Model file for the job. Use its own axes, mm. A direction names the side the tool comes from. Coordinates: 2 decimals unless noted, no trailing zeros. Loops run counter-clockwise (first coordinate to the right, second up) from the corner with the lowest first, then second, coordinate; pieces in that order, holes last. Notation, with made-up numbers: (21.5, 29.5) - (68.5, 29.5) arc R31 ccw to (68.5, 65.5) - close; hole circle Ø8 at (16.25, -38.75). An arc over 180 degrees is marked (long way). Write each question's results on one line, items separated by ' | '. Start each with the question number.
```python
from build123d import *

# Parameters (mm, degrees)
BOSS_EXTRUDE1_DEPTH = 32
SKETCH2_R           = 2.1
CUT_EXTRUDE1_DEPTH  = 35.76550014
SKETCH3_R           = 1.740904785
BOSS_EXTRUDE2_DEPTH = 0.1
SKETCH4_R           = 3.5
BOSS_EXTRUDE3_DEPTH = 4
SKETCH5_R           = 2.5
BOSS_EXTRUDE4_DEPTH = 62
FILLET1_R           = 0.2
FILLET2_R           = 0.5
SKETCH6_W           = 7.2
SKETCH6_H           = 30
CUT_EXTRUDE2_DEPTH  = 19
SKETCH7_W           = 16.27166032
SKETCH7_H           = 23.629900988
CUT_EXTRUDE3_DEPTH  = 74.5
SKETCH8_R           = 1.9
CUT_EXTRUDE4_DEPTH  = 17.5
SKETCH9_R           = 3.1
SKETCH9_R_2         = 2.1
BOSS_EXTRUDE5_DEPTH = 7.2


with BuildPart() as part:
    # Sketch1 → Boss-Extrude1 (new body)
    with BuildSketch(Plane(origin=(0, 0, 0), x_dir=(1, 0, 0), z_dir=(0, 1, 0))):
        Polygon((2, -10), (4.6, -10), (4.6, 10), (-4.6, 10), (-4.6, -10), (-2, -10), (-2, -9.7), (2, -9.7), align=None)
    extrude(amount=BOSS_EXTRUDE1_DEPTH)

    # Sketch2 → Cut-Extrude1 (cut, through all)
    with BuildSketch(Plane(origin=(4.6, 0, 0), x_dir=(0, 0, -1), z_dir=(1, 0, 0))):
        with Locations((5, 26)):
            Circle(SKETCH2_R)
        with Locations((5, 6)):
            Circle(SKETCH2_R)
    extrude(amount=-CUT_EXTRUDE1_DEPTH, mode=Mode.SUBTRACT)

    # Sketch3 → Boss-Extrude2 (add)
    with BuildSketch(Plane(origin=(0, 0, -10), x_dir=(-1, 0, 0), z_dir=(0, 0, -1))):
        with Locations((0, 18.961857961)):
            Circle(SKETCH3_R)
    extrude(amount=BOSS_EXTRUDE2_DEPTH)

    # Sketch4 → Boss-Extrude3 (add)
    with BuildSketch(Plane.XZ):
        with Locations(Location((0, 0, 0), (0, 0, 270))):
            Circle(SKETCH4_R)
    extrude(amount=BOSS_EXTRUDE3_DEPTH)

    # Sketch5 → Boss-Extrude4 (add)
    with BuildSketch(Plane.XZ.offset(4)):
        with Locations(Location((0, 0, 0), (0, 0, 270))):
            Circle(SKETCH5_R)
    extrude(amount=BOSS_EXTRUDE4_DEPTH)

    # Fillet1
    fillet1_edges = [part.edges().sort_by_distance(p)[0] for p in [
        (0, -4, 3.5),
    ]]
    fillet(fillet1_edges, radius=FILLET1_R)

    # Fillet2
    fillet2_edges = [part.edges().sort_by_distance(p)[0] for p in [
        (0, 0, -10),
        (0, 32, -10),
    ]]
    fillet(fillet2_edges, radius=FILLET2_R)

    # Sketch6 → Cut-Extrude2 (cut)
    with BuildSketch(Plane.XY.offset(10)):
        with Locations((0, 16)):
            Rectangle(SKETCH6_W, SKETCH6_H)
    extrude(amount=-CUT_EXTRUDE2_DEPTH, mode=Mode.SUBTRACT)

    # Sketch7 → Cut-Extrude3 (cut)
    with BuildSketch(Plane.XZ):
        with Locations((-4.097079532, -5.79987022)):
            Rectangle(SKETCH7_W, SKETCH7_H)
    extrude(amount=CUT_EXTRUDE3_DEPTH, mode=Mode.SUBTRACT)

    # Sketch8 → Cut-Extrude4 (cut)
    with BuildSketch(Plane.XZ):
        with Locations(Location((0, 0, 0), (0, 0, 270))):
            Circle(SKETCH8_R)
    extrude(amount=-CUT_EXTRUDE4_DEPTH, mode=Mode.SUBTRACT)

    # Sketch9 → Boss-Extrude5 (add)
    # profile 1 of 2: a face of its own
    with BuildSketch(Plane.ZY.offset(-3.6)):
        with Locations(Location((-5, 26, 0), (0, 0, 90))):
            Circle(SKETCH9_R)
        with Locations(Location((-5, 26, 0), (0, 0, 180))):
            Circle(SKETCH9_R_2, mode=Mode.SUBTRACT)
    # profile 2 of 2: a face of its own
    with BuildSketch(Plane.ZY.offset(-3.6)):
        with Locations(Location((-5, 6, 0), (0, 0, 90))):
            Circle(SKETCH9_R)
        with Locations(Location((-5, 6, 0), (0, 0, 180))):
            Circle(SKETCH9_R_2, mode=Mode.SUBTRACT)
    extrude(amount=BOSS_EXTRUDE5_DEPTH)


solid = part.part
```
Q1. Which spindle directions (+Z, -Z, +X, -X, +Y, -Y) get a long thin tool onto all of the face, cutting with end or side? Do faces 5 (the flat face through (0, 19, -10.1)), 6 (the flat face through (0, 16, -9)), 7 (the flat face through (0, 0.5, 9.7)), 8 (the flat face through (0, 31, 1)). Say none if no direction does.
Q2. Cut at C-C (z = -5). List the corners of the cut face in (x, y).
Q3. Pin check, flat tips, straight feed: pin 1 (3 mm diameter, centred on x = 2, y = 25, fed in from -Z); pin 2 (2 mm diameter, centred on x = 1, y = 7.5, fed in from +Z). Stop position of each tip, or through.
Q4. Cut at A-A (y = 6). List the corners of the cut face in (x, z), and give its area (3 significant figures).
Q5. Cut at B-B (x = 0). List the corners of the cut face in (y, z), and give its area (3 significant figures).
Q6. Cut at D-D (y = 22). List the corners of the cut face in (x, z), and give its area (3 significant figures).
Q7. Drill centre lines: L1, parallel to Y at x = 4.1, z = -5; L2, parallel to X at y = 23.5, z = 3.75; L3, parallel to Y at x = 2.75, z = -3.5. Where is each one in solid material? Low to high. Write a range as from..to.
Q8. Mould opens along Z. For faces 1 (the cylindrical face through (-0.728, 0.493, -1.755)), 2 (the flat face through (-4.6, 16, 0)), 3 (the flat face through (-4, 16, 10)), 4 (the flat face through (0, 16, -10)) say: +Z half, -Z half, draft (parallel to the pull), parting line (faces both ways), or undercut.
Check result:
1) face 5: -Z, +X, -X, +Y, -Y | face 6: none | face 7: +Z, +Y, -Y | face 8: +Z
2) outline: (-4.6, 0) - (4.6, 0) - (4.6, 3.9) - (-4.6, 3.9) - close; (-4.6, 8.1) - (4.6, 8.1) - (4.6, 23.9) - (-4.6, 23.9) - close; (-4.6, 28.1) - (4.6, 28.1) - (4.6, 32) - (-4.6, 32) - close; hole (-3.6, 1) - (3.6, 1) - (3.6, 2.9) - (-3.6, 2.9) - close; hole (-3.6, 9.1) - (3.6, 9.1) - (3.6, 22.9) - (-3.6, 22.9) - close; hole (-3.6, 29.1) - (3.6, 29.1) - (3.6, 31) - (-3.6, 31) - close
3) pin 1: z = -10 | pin 2: z = -1.94
4) outline: (-4.6, -10) - (4.6, -10) - (4.6, -7.1) - (-4.6, -7.1) - close; (-4.6, -2.9) - (4.6, -2.9) - (4.6, 10) - (3.6, 10) - (3.6, -1.9) - (-3.6, -1.9) - (-3.6, 10) - (-4.6, 10) - close; hole (-3.6, -9) - (3.6, -9) - (3.6, -8.1) - (-3.6, -8.1) - close | area: 53.2 mm²
5) outline: (0, -9.5) arc R0.5 ccw to (0.5, -10) - (17.22, -10) - (17.22, -10.1) - (20.7, -10.1) - (20.7, -10) - (31.5, -10) arc R0.5 ccw to (32, -9.5) - (32, 9.7) - (31, 9.7) - (31, -9) - (1, -9) - (1, -1.9) - (0, -1.9) - close; (0, 1.9) - (1, 1.9) - (1, 9.7) - (0, 9.7) - close; circle Ø6.2 at (6, -5); circle Ø6.2 at (26, -5); hole circle Ø4.2 at (6, -5); hole circle Ø4.2 at (26, -5) | area: 98.5 mm²
6) outline: (-4.6, -10) - (4.6, -10) - (4.6, 10) - (3.6, 10) - (3.6, -9) - (-3.6, -9) - (-3.6, 10) - (-4.6, 10) - close | area: 47.2 mm²
7) L1: 0..3.9, 8.1..23.9, 28.1..32 | L2: -4.6..-3.6, 3.6..4.6 | L3: 0..1, 3.29..4.53, 7.47..8.71, 23.29..24.53, 27.47..28.71, 31..32
8) face 1: undercut | face 2: draft | face 3: +Z half | face 4: -Z half
